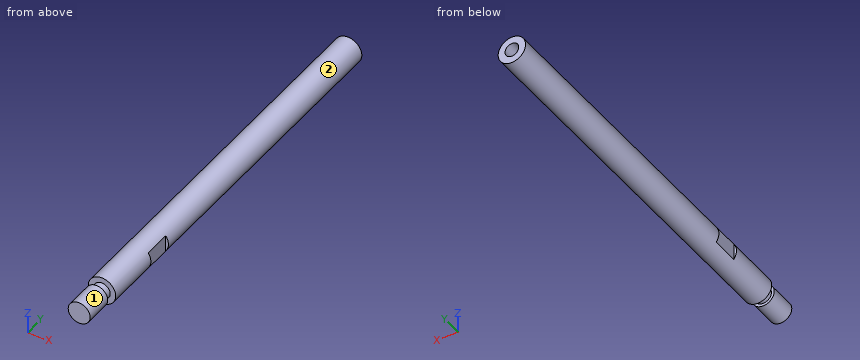
```python
from build123d import *

# Parameters (mm, degrees)
CUT_EXTRUDE1_DEPTH      = 140.008995048
CUT_EXTRUDE1_DEPTH_BACK = 140.008995048
SKETCH2_W               = 1
SKETCH2_H               = 10
M6_TAPPED_HOLE1_D       = 5
M6_TAPPED_HOLE1_DEPTH   = 12
M6_TAPPED_HOLE1_TIP     = 1.502151548


with BuildPart() as part:
    # Sketch1 → Revolve1 (revolve)
    with BuildSketch(Plane.XY):
        Polygon((0, 14.170965918), (0, -138.829034082), (-4, -138.829034082), (-4, -128.829034082), (-3, -128.829034082), (-3, -125.829034082), (-5, -125.829034082), (-5, 14.170965918), align=None)
    revolve(axis=Axis((0, 14.170965918, 0), (0, -1, 0)))

    # Sketch2 → Cut-Extrude1 (cut, two sides: drawn at the far end of the back side and taken through both)
    with BuildSketch(Plane.XY.offset(-CUT_EXTRUDE1_DEPTH_BACK)):
        with Locations((-4.5, -100.829034082)):
            Rectangle(SKETCH2_W, SKETCH2_H)
        with Locations((4.5, -100.829034082)):
            Rectangle(SKETCH2_W, SKETCH2_H)
    extrude(amount=CUT_EXTRUDE1_DEPTH + CUT_EXTRUDE1_DEPTH_BACK, mode=Mode.SUBTRACT)

    # M6 Tapped Hole1
    with Locations(Plane(origin=(0, 14.170965918, 0), x_dir=(1, 0, 0), z_dir=(0, 1, 0))):
        with Locations((0, 0)):
            Hole(M6_TAPPED_HOLE1_D / 2, depth=M6_TAPPED_HOLE1_DEPTH)
            with Locations((0, 0, -(M6_TAPPED_HOLE1_DEPTH + M6_TAPPED_HOLE1_TIP / 2))):  # 118° drill point
                Cone(0, M6_TAPPED_HOLE1_D / 2, M6_TAPPED_HOLE1_TIP, mode=Mode.SUBTRACT)


solid = part.part
```
Geometry check sheet. Reference: the model listing, model coordinates, mm. Face numbers are marked on the shaded views. A direction names the side the tool comes from. Give positions to 0.01 mm unless a question says otherwise; leave off trailing zeros. Order: outer loops, then holes, each group sorted by start corner. A loop starts at its lowest first (then second) coordinate and runs counter-clockwise, first axis right, second up.
1. Gauge pin test, flat ends, axial feed: pin 1 Ø3 at (y, z) = (-103.5, -1) entering from -X; pin 2 Ø1.5 at (y, z) = (-116.5, 2) entering from +X; pin 3 Ø0.8 at (x, z) = (-4.5, 0) entering from -Y. Record the tip position at first contact, or that the pin passes through.
2. Thickness scan on L1, parallel to Z at x = 0, y = 10.75; L2, parallel to Y at x = -2, z = -2.5; L3, parallel to Y at x = 4.25, z = -2.25. Record the ranges inside material, lowest first.
3. Section check A-A, the plane y = -115.5. Enter the section's corners in (x, z).
4. Access from +Z, -Z, +X, -X, +Y, -Y to the whole of each face (thin tool, end or side, straight path). Record for the marked faces 1 and 2.
Values follow:
1. pin 1: stops at x = -4
1. pin 2: stops at x = 4.84
1. pin 3: stops at y = -125.83
2. L1: z = -5 to -2.5, 2.5 to 5
2. L2: y = -138.83 to -128.83, -125.83 to 14.17
2. L3: y = -125.83 to -105.83, -95.83 to 14.17
3. outline: circle Ø10 at (0, 0)
4. face 1: -Y
4. face 2: +Y, -Y
